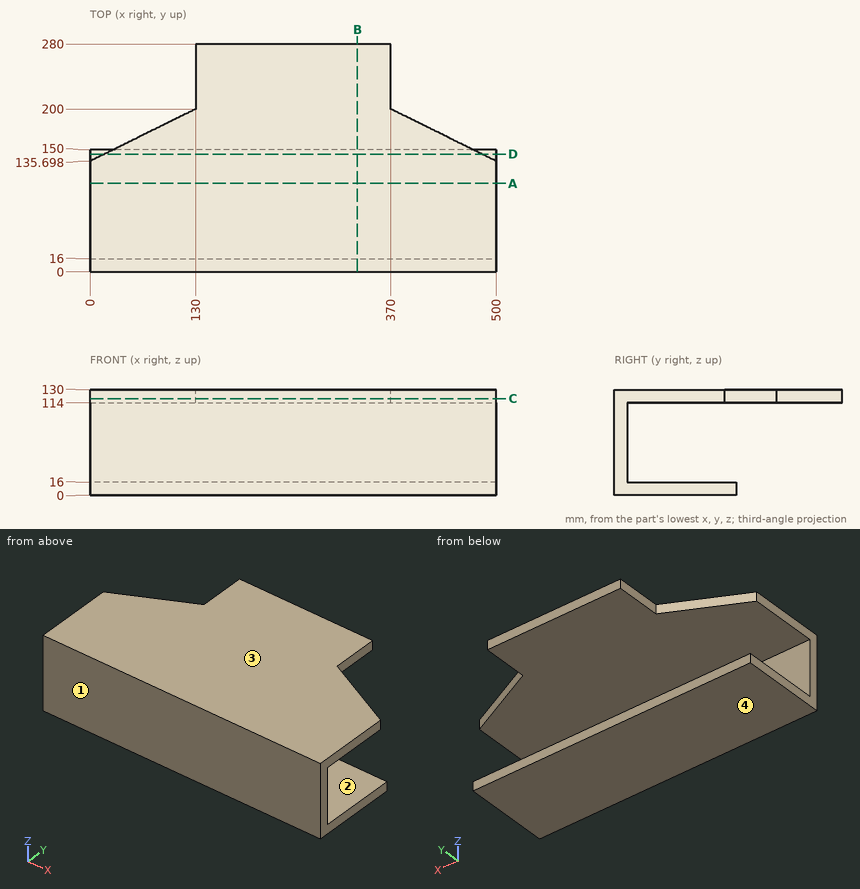
Check sheet for the drawn part. Datum: minimum x, y, z corner. Units: mm. Coordinates: 2 decimals unless noted, no trailing zeros. Order: outer loops, then holes, each group sorted by start corner. A loop starts at its lowest first (then second) coordinate and runs counter-clockwise, first axis right, second up. Notation, with made-up numbers: (36, -26.75) -> (87, -26.75) arc R10 ccw to (87, -20.75) -> close; hole circle Ø6 at (51.25, 22). An arc over 180 degrees is marked (long way). Write each question's results on one line, items separated by ' | '. Start each with the question number.
1) Section check A-A (y = 108.5). Enter the section's corners in (x, z).
2) Material ranges on line 1 along Z through (x, y) = (86.5, 39.5); line 2 along Z through (x, y) = (180, 242.5); line 3 along Y through (x, z) = (97, 62), recorded low to high.
3) Section check D-D (y = 144.5). Enter the section's corners in (x, z).
4) Depth check by flat-ended pin: pin 1 (1 mm diameter, centred on x = 146, y = 160.5, fed in from -Z); pin 2 (13 mm diameter, centred on y = 239.5, z = 121.5, fed in from -X); pin 3 (1 mm diameter, centred on x = 359.5, z = 43, fed in from +Y). Enter the tip coordinate at first touch or a pass-through.
5) Section check B-B (x = 329). Enter the section's corners in (y, z).
6) Section check C-C (z = 119). Enter the section's corners in (x, y), and give its area (3 significant figures).
7) Draft check along Z on the marked faces 1, 2, 3 and 4. Enter one of: pulls with the +Z half, pulls with the -Z half, needs draft (parallel to the pull), parting line crosses it, or undercut.
Checked values:
1) outline: (0, 0) -> (500, 0) -> (500, 16) -> (0, 16) -> close; (0, 114) -> (500, 114) -> (500, 130) -> (0, 130) -> close
2) line 1: 0 to 16, 114 to 130 | line 2: 114 to 130 | line 3: 0 to 16
3) outline: (0, 0) -> (500, 0) -> (500, 16) -> (0, 16) -> close; (17.8, 114) -> (482.2, 114) -> (482.2, 130) -> (17.8, 130) -> close
4) pin 1: z = 114 | pin 2: x = 130 | pin 3: y = 16
5) outline: (0, 0) -> (150, 0) -> (150, 16) -> (16, 16) -> (16, 114) -> (280, 114) -> (280, 130) -> (0, 130) -> close
6) outline: (0, 0) -> (500, 0) -> (500, 135.7) -> (370, 200) -> (370, 280) -> (130, 280) -> (130, 200) -> (0, 135.7) -> close | area: 111,000 mm²
7) face 1: needs draft | face 2: undercut | face 3: pulls with the +Z half | face 4: pulls with the -Z half
